Check sheet for the modelled part. Datum: model origin and axes. Units: mm. A direction names the side the tool comes from. Round coordinates to 2 decimals unless told otherwise and drop trailing zeros. Write each loop counter-clockwise with the first axis right and the second up, starting at its lowest first coordinate (ties: lowest second). Pieces come first, ordered by that corner, then holes. Notation, with made-up numbers: (83, 17) -> (92, 17) arc R4 cw to (92, 24) -> close; hole circle Ø10 at (-8.5, 17). An arc over 180 degrees is marked (long way). Answer as a JSON object with one key per item and string values. Group by question number.
```python
from build123d import *

# Parameters (mm, degrees)
CUT_EXTRUDE1_DEPTH      = 135.169668703
CUT_EXTRUDE1_DEPTH_BACK = 135.169668703
SKETCH2_R               = 3
CUT_EXTRUDE2_DEPTH      = 135.169668803
CUT_EXTRUDE2_DEPTH_BACK = 8
SKETCH3_R               = 3
SKETCH4_R               = 1.5
CUT_EXTRUDE3_DEPTH      = 50
CHAMFER1_SIZE           = 1.5
CHAMFER1_SIZE2          = 0.866025404
CHAMFER2_SIZE           = 1


with BuildPart() as part:
    # Sketch1 → Revolve1 (revolve)
    with BuildSketch(Plane.XY, mode=Mode.PRIVATE) as revolve1_sk:
        Polygon((0, 0), (0, 8), (12.5, 8), (12.5, 7), (15, 7), (15, 9), (46.5, 9), (46.5, 8.5), (48.5, 8.5), (48.5, 12.5), (53, 12.5), (53, 7.5), (55, 7.5), (55, 8), (133, 8), (133, 0), align=None)
    revolve(revolve1_sk.sketch.rotate(Axis((133, 0, 0), (-1, 0, 0)), 90), axis=Axis((133, 0, 0), (-1, 0, 0)))

    # Sketch2 → Cut-Extrude1 (cut, two sides: drawn at the far end of the back side and taken through both)
    with BuildSketch(Plane.XY.offset(-CUT_EXTRUDE1_DEPTH_BACK)):
        with Locations((117.5, 0)):
            Circle(SKETCH2_R)
    extrude(amount=CUT_EXTRUDE1_DEPTH + CUT_EXTRUDE1_DEPTH_BACK, mode=Mode.SUBTRACT)

    # Sketch3 → Cut-Extrude2 (cut, two sides: drawn at the far end of the back side and taken through both)
    with BuildSketch(Plane.ZY.offset(-CUT_EXTRUDE2_DEPTH_BACK)):
        with Locations(Location((0, 0, 0), (0, 0, 180))):
            Circle(SKETCH3_R)
    extrude(amount=CUT_EXTRUDE2_DEPTH + CUT_EXTRUDE2_DEPTH_BACK, mode=Mode.SUBTRACT)

    # Sketch4 → Cut-Extrude3 (cut)
    with BuildSketch(Plane.ZY.offset(-8)):
        Circle(SKETCH4_R)
    extrude(amount=-CUT_EXTRUDE3_DEPTH, mode=Mode.SUBTRACT)

    # Chamfer1
    chamfer1_edges = [part.edges().sort_by_distance(p)[0] for p in [
        (0, 0, 3),
    ]]
    chamfer1_side = [part.faces().sort_by_distance(p)[0] for p in [
        (4, 0, 3),
    ]]
    chamfer(chamfer1_edges, length=CHAMFER1_SIZE, length2=CHAMFER1_SIZE2, reference=chamfer1_side[0])

    # Chamfer2
    chamfer2_edges = [part.edges().sort_by_distance(p)[0] for p in [
        (133, 0, 8),
        (0, 0, 8),
    ]]
    chamfer(chamfer2_edges, length=CHAMFER2_SIZE)

    # Sketch5 → Cut-Revolve1 (revolve, cut)
    with BuildSketch(Plane.XY):
        with BuildLine():
            Line((58, 1.5), (58, -1.5))
            ThreePointArc((58, -1.5), (59.5, 0), (58, 1.5))
        make_face()
    revolve(axis=Axis((58, 1.5, 0), (0, -1, 0)), mode=Mode.SUBTRACT)


solid = part.part
```
(1) Section check B-B on x = 66. Record the cut outline in (y, z), then the cut area to 3 significant figures.
(2) Section check C-C on x = 117.5. Record the cut outline in (y, z), then the cut area to 3 significant figures.
(3) Access from +Z, -Z, +X, -X, +Y, -Y to the whole of each face (thin tool, end or side, straight path). Record for faces 4 (the cylindrical face through (50.782, -3.755, -11.923)), 5 (the cylindrical face through (54.014, -6.324, -4.032)), 6 (the flat face through (8, 1.3, -1.3)).
(4) Release check for a two-part mould opening along Y. For faces 1 (the flat face through (12.5, 6, -4)), 2 (the cylindrical face through (32.65, 0.07, -1.5)), 3 (the cylindrical face through (30.97, -6.083, 6.633)) record: pulls with the +Y half, pulls with the -Y half, needs draft (parallel to the pull), parting line crosses it, or undercut.
(5) Go/stop test with flat-tipped pins: pin 1 Ø3 at (y, z) = (-9, 4.5) entering from +X; pin 2 Ø10 at (x, y) = (52, 6.5) entering from -Z; pin 3 Ø3.5 at (x, y) = (117.5, 0) entering from -Z; pin 4 Ø6 at (x, y) = (115, -7.5) entering from -Z. Record where each tip stops, or that it passes through.
(6) Scan lines: line 1 along Y through (x, z) = (36.5, 0); line 2 along Y through (x, z) = (5, 0); line 3 along X through (y, z) = (3, -8.25). Record each from-to range of solid material in increasing order.
(7) Section check A-A on x = 30.5. Record the cut outline in (y, z).
Data:
{
 "1": {"outline": "circle Ø16 at (0, 0)", "area": "201 mm²"},
 "2": {"outline": "(-3, -7.42) -> (-3, 7.42) arc R8 ccw to start; (3, -7.42) arc R8 ccw to (3, 7.42) -> close", "area": "107 mm²"},
 "3": {"face 4": "+X, -X", "face 5": "none", "face 6": "-X"},
 "4": {"face 1": "needs draft", "face 2": "undercut", "face 3": "parting line crosses it"},
 "5": {"pin 1": "stops at x = 53", "pin 2": "stops at z = -12.41", "pin 3": "passes through", "pin 4": "stops at z = -6.61"},
 "6": {"line 1": "y = -9 to -1.5, 1.5 to 9", "line 2": "y = -8 to -3, 3 to 8", "line 3": "x = 15 to 46.5, 48.5 to 53"},
 "7": {"outline": "circle Ø18 at (0, 0); hole circle Ø3 at (0, 0)"}
}
